from build123d import *

# Parameters (mm, degrees)
BOSS_EXTRUDE1_DEPTH = 9


with BuildPart() as part:
    # Sketch1 → Boss-Extrude1 (new body)
    with BuildSketch(Plane(origin=(0, 0, 0), x_dir=(-1, 0, 0), z_dir=(0, 1, 0))):
        with BuildLine():
            Line((-145.613884922, 900), (-145.613884922, 500))
            ThreePointArc((-145.613884922, 500), (-138.461432518, 482.732452403), (-121.193884922, 475.58))
            Line((-121.193884922, 475.58), (78.806115078, 475.58))
            ThreePointArc((78.806115078, 475.58), (99.138824975, 486.475307462), (101.328117521, 509.439057473))
            Line((101.328117521, 509.439057473), (37.4278997, 661.90776168))
            ThreePointArc((37.4278997, 661.90776168), (37.336543074, 667.86452336), (41.387455782, 672.23275664))
            Line((41.387455782, 672.23275664), (75.344343138, 688.282934243))
            ThreePointArc((75.344343138, 688.282934243), (82.766115078, 700), (75.344343138, 711.717065757))
            Line((75.344343138, 711.717065757), (41.387455782, 727.76724336))
            ThreePointArc((41.387455782, 727.76724336), (37.336543074, 732.13547664), (37.4278997, 738.09223832))
            Line((37.4278997, 738.09223832), (101.328117521, 890.560942527))
            ThreePointArc((101.328117521, 890.560942527), (99.138824975, 913.524692538), (78.806115078, 924.42))
            Line((78.806115078, 924.42), (-121.193884922, 924.42))
            ThreePointArc((-121.193884922, 924.42), (-138.461432518, 917.267547597), (-145.613884922, 900))
        make_face()
        with BuildLine():
            Line((-144.113884922, 900), (-144.113884922, 500))
            ThreePointArc((-144.113884922, 500), (-137.400772347, 483.793112575), (-121.193884922, 477.08))
            Line((-121.193884922, 477.08), (78.806115078, 477.08))
            ThreePointArc((78.806115078, 477.08), (97.889887021, 487.306062532), (99.944702137, 508.859262788))
            Line((99.944702137, 508.859262788), (36.044484316, 661.327966995))
            ThreePointArc((36.044484316, 661.327966995), (35.935998324, 668.40162149), (40.746457164, 673.58889851))
            Line((40.746457164, 673.58889851), (74.70334452, 689.639076113))
            ThreePointArc((74.70334452, 689.639076113), (81.266115078, 700), (74.70334452, 710.360923887))
            Line((74.70334452, 710.360923887), (40.746457164, 726.41110149))
            ThreePointArc((40.746457164, 726.41110149), (35.935998324, 731.59837851), (36.044484316, 738.672033005))
            Line((36.044484316, 738.672033005), (99.944702137, 891.140737212))
            ThreePointArc((99.944702137, 891.140737212), (97.889887021, 912.693937468), (78.806115078, 922.92))
            Line((78.806115078, 922.92), (-121.193884922, 922.92))
            ThreePointArc((-121.193884922, 922.92), (-137.400772347, 916.206887425), (-144.113884922, 900))
        make_face(mode=Mode.SUBTRACT)
    extrude(amount=BOSS_EXTRUDE1_DEPTH)


solid = part.part
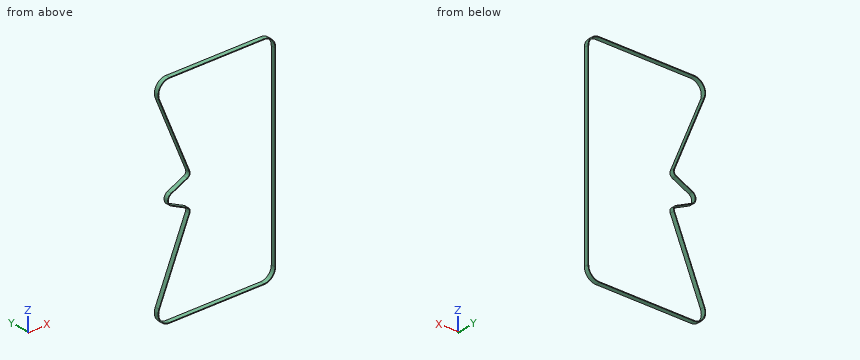
Can you work these out from the model? Positions are in its coordinate system, mm. Give positions to 0.01 mm unless a question says otherwise; leave off trailing zeros. Loops run counter-clockwise (first coordinate to the right, second up) from the corner with the lowest first, then second, coordinate; pieces in that order, holes last. Notation, with made-up numbers: (88.5, 88) - (117.5, 88) arc R19 ccw to (117.5, 102) - close; hole circle Ø2 at (59, 44.25). An arc over 180 degrees is marked (long way). Answer as a JSON object with one key per item and string values.
Q1. If I drill on L1, parallel to Z at x = 36.5, y = 8.25; L2, parallel to Z at x = -71.5, y = 4.75; L3, parallel to Z at x = -42.5, y = 5.5, over which ranges is the centre line in solid material (lowest first)?
Geometry says:
{"L1": "475.58 to 477.08, 922.92 to 924.42", "L2": "475.58 to 477.08, 576.73 to 580.61, 686.47 to 688.12, 711.88 to 713.53, 819.39 to 823.27, 922.92 to 924.42", "L3": "475.58 to 477.08, 645.92 to 649.81, 672.76 to 674.42, 725.58 to 727.24, 750.19 to 754.08, 922.92 to 924.42"}
Q2. Imagine slicing it at A-A on x = 3. Write out the boundary of the cut face in (y, z), plus the area to 3 significant figures.
Geometry says:
{"outline": "(0, 475.58) - (9, 475.58) - (9, 477.08) - (0, 477.08) - close; (0, 922.92) - (9, 922.92) - (9, 924.42) - (0, 924.42) - close", "area": "27.0 mm²"}
Q3. Imagine slicing it at D-D on z = 579. Write out the boundary of the cut face in (x, y).
Geometry says:
{"outline": "(-72.17, 0) - (-70.55, 0) - (-70.55, 9) - (-72.17, 9) - close; (144.11, 0) - (145.61, 0) - (145.61, 9) - (144.11, 9) - close"}
Q4. Will this pin go through, and if not, where does the flat tip stop? P1, Ø4.5, axis at y = 2.5, z = 677, coming from the -X side.
Geometry says:
{"P1": "x = -56.23"}
Q5. Imagine slicing it at B-B on y = 6.25. Write out the boundary of the cut face in (x, z), plus the area to 3 significant figures.
Geometry says:
{"outline": "(-101.33, 509.44) arc R24.42 ccw to (-78.81, 475.58) - (121.19, 475.58) arc R24.42 ccw to (145.61, 500) - (145.61, 900) arc R24.42 ccw to (121.19, 924.42) - (-78.81, 924.42) arc R24.42 ccw to (-101.33, 890.56) - (-37.43, 738.09) arc R8 cw to (-41.39, 727.77) - (-75.34, 711.72) arc R12.96 ccw to (-75.34, 688.28) - (-41.39, 672.23) arc R8 cw to (-37.43, 661.91) - close; hole (-99.94, 508.86) arc R22.92 ccw to (-78.81, 477.08) - (121.19, 477.08) arc R22.92 ccw to (144.11, 500) - (144.11, 900) arc R22.92 ccw to (121.19, 922.92) - (-78.81, 922.92) arc R22.92 ccw to (-99.94, 891.14) - (-36.04, 738.67) arc R9.5 cw to (-40.75, 726.41) - (-74.7, 710.36) arc R11.46 ccw to (-74.7, 689.64) - (-40.75, 673.59) arc R9.5 cw to (-36.04, 661.33) - close", "area": "2,140 mm²"}
Q6. Imagine slicing it at C-C on x = -47.5. Write out the boundary of the cut face in (y, z), plus the area to 3 significant figures.
Geometry says:
{"outline": "(0, 475.58) - (9, 475.58) - (9, 477.08) - (0, 477.08) - close; (0, 633.99) - (9, 633.99) - (9, 637.88) - (0, 637.88) - close; (0, 675.12) - (9, 675.12) - (9, 676.78) - (0, 676.78) - close; (0, 723.22) - (9, 723.22) - (9, 724.88) - (0, 724.88) - close; (0, 762.12) - (9, 762.12) - (9, 766.01) - (0, 766.01) - close; (0, 922.92) - (9, 922.92) - (9, 924.42) - (0, 924.42) - close", "area": "127 mm²"}
